Check sheet for the drawn part. Datum: minimum x, y, z corner. Units: mm. A direction names the side the tool comes from. Round coordinates to 2 decimals unless told otherwise and drop trailing zeros.
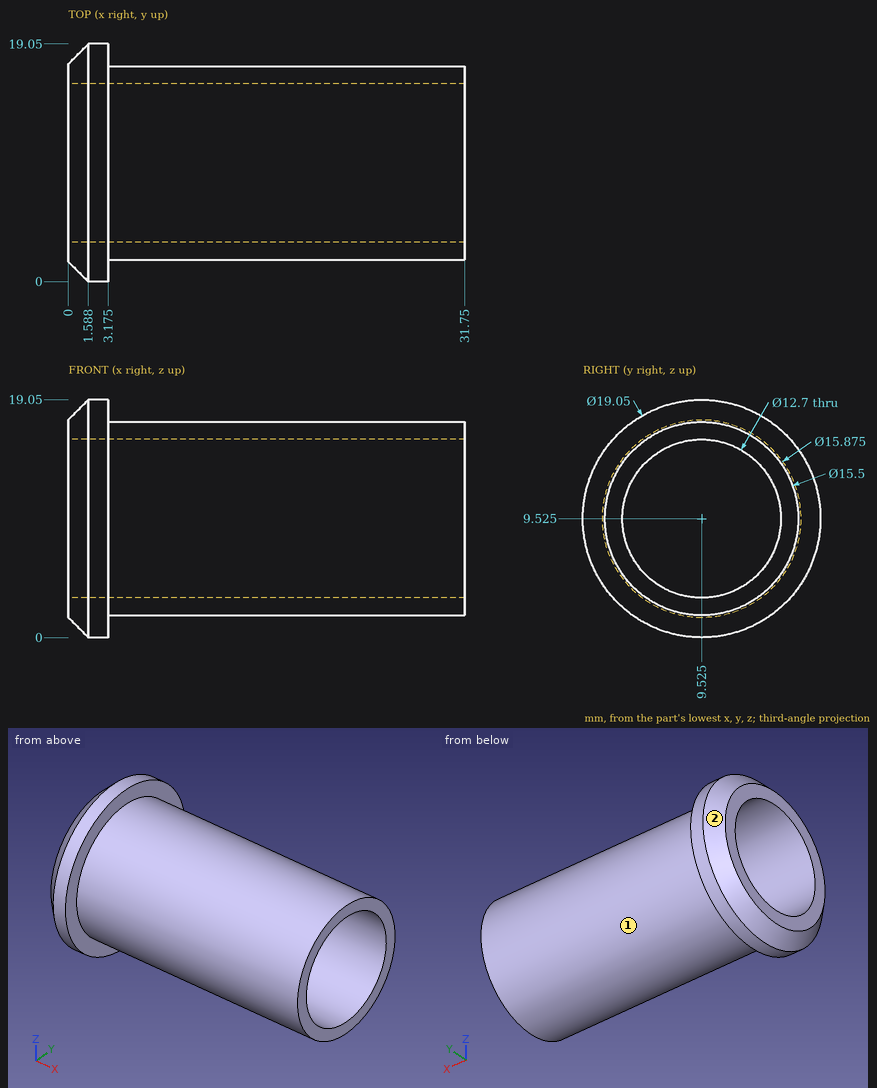
Q1. Depth check by flat-ended pin: P1, Ø6, axis at y = 13, z = 11.5, coming from the +X side; P2, Ø6, axis at x = 23, z = 5, coming from the +Y side; P3, Ø5, axis at x = 5, z = 3.5, coming from the +Y side (1 decimal); P4, Ø1, axis at x = 21, z = 16, coming from the -Y side. Enter the tip coordinate at first touch or a pass-through.
Recorded:
P1: stops at x = 31.75
P2: stops at y = 17.12
P3: stops at y = 18
P4: stops at y = 4.59
Q2. Tool access check on the marked faces 1 and 2. Record the directions out of +Z, -Z, +X, -X, +Y, -Y that give a thin tool (end or side, any length) a straight path to the whole face; none if there is none.
Recorded:
face 1: +X
face 2: -X
Q3. Material ranges on line 1 along Z through (x, y) = (17.5, 9.25); line 2 along Y through (x, z) = (26, 5) (1 decimal); line 3 along Y through (x, z) = (18.5, 8), recorded low to high.
Recorded:
line 1: z = 1.78 to 3.18, 15.87 to 17.27
line 2: y = 3.2 to 5.1, 14 to 15.8
line 3: y = 1.93 to 3.36, 15.69 to 17.12
